from build123d import *

# Parameters (mm, degrees)
BOSS_EXTRUDE1_DEPTH = 62
SWEEP1_PROFILE_R    = 3
FILLET3_R           = 2


with BuildPart() as part:
    # Sketch1 → Boss-Extrude1 (new body)
    with BuildSketch(Plane(origin=(0, 0, 0), x_dir=(1, 0, 0), z_dir=(0, 1, 0))):
        with BuildLine():
            Line((0, 5), (-20, 5))
            Line((-20, 5), (-20, 3))
            Line((-20, 3), (0, 3))
            ThreePointArc((0, 3), (1.826284287, -2.380060021), (-2.897777479, 0.776457135))
            Line((-2.897777479, 0.776457135), (-4.829629131, 1.294095226))
            ThreePointArc((-4.829629131, 1.294095226), (3.043807145, -3.966766701), (0, 5))
        make_face()
    extrude(amount=BOSS_EXTRUDE1_DEPTH)

    # Sweep1: sweep along a path in Sketch2
    with BuildLine(Plane.XY) as sweep1_path:
        Line((0, 78.5), (0, 0))
        Line((0, 0), (0, -11.5))
        ThreePointArc((0, -11.5), (-1.464466094, -15.035533906), (-5, -16.5))
        Line((-5, -16.5), (-20, -16.5))
    # Sweep1 profile (on start of the path) → Sweep1 (sweep)
    with BuildSketch(Plane(origin=(0, 78.5, 0), x_dir=(0, 0, -1), z_dir=(0, -1, 0))):
        Circle(SWEEP1_PROFILE_R)
    sweep(path=sweep1_path.line)

    # Fillet3
    fillet3_edges = [part.edges().sort_by_distance(p)[0] for p in [
        (-20, 62, -4),
        (-20, 0, -4),
    ]]
    fillet(fillet3_edges, radius=FILLET3_R)


solid = part.part
Model file for the job. Use its own axes, mm. A direction names the side the tool comes from. Give positions to 0.01 mm unless a question says otherwise; leave off trailing zeros. Write each loop counter-clockwise with the first axis right and the second up, starting at its lowest first coordinate (ties: lowest second). Pieces come first, ordered by that corner, then holes. Notation, with made-up numbers: M -1,83.25 L 6,83.25 A29 cw 6,121.25 Z; hole C 49.25,45.25 d9. An arc over 180 degrees is marked long. One line per item, written item: value. Start each with the question number.
Q1. 3-axis set-ups, long thin cutter, end or side, ignore diameter. For faces 1 (the cylindrical face through (-12.6, -13.57, 0.65)), 2 (the flat face through (-20, 31, -4)), 3 (the cylindrical face through (3, 31, 4)), 4 (the cylindrical face through (-1.15, 42.87, -2.77)): which of +Z, -Z, +X, -X, +Y, -Y reach the whole face in a straight line?
Q2. Probe probe 1 along Y at (x, z) = (0.5, 3.75); probe 2 along Z at (x, y) = (-8.75, 39); probe 3 along Z at (x, y) = (-2.5, 35). List the from-to ranges inside material, lowest first. Write a range as [from, to].
Q3. Saw through at A-A, the plane x = -16.5. Write the cut outline in (y, z), plus the area to 3 significant figures.
Q4. Drop flat-ended pins along their axis: pin 1 Ø1.5 at (x, z) = (-7.5, -1.5) entering from +Y; pin 2 Ø3 at (x, z) = (-6, 2) entering from +Y; pin 3 Ø1 at (x, z) = (-11, -2) entering from -Y. Give the stop position or say it passes through.
Q5. Saw through at B-B, the plane y = 13. Write the cut outline in (x, z), plus the area to 3 significant figures.
Output values:
1. face 1: -X
1. face 2: +Z, -Z, -X, +Y, -Y
1. face 3: +Y
1. face 4: none
2. probe 1: y = [0, 62]
2. probe 2: z = [-5, -3]
2. probe 3: z = [-5, -3], [-1.66, 4.33]
3. outline: C -16.5,0 d6; M 0,-5 L 62,-5 L 62,-3 L 0,-3 Z
3. area: 152 mm²
4. pin 1: stops at y = -13.6
4. pin 2: stops at y = 62
4. pin 3: stops at y = -19.1
5. outline: M -20,-5 L 0,-5 A5 ccw long -4.83,-1.29 L -2.9,-0.78 A3 ccw 0,-3 L -20,-3 Z
5. area: 108 mm²
